from build123d import *

# Parameters (mm, degrees)
CUT_EXTRUDE_1_DEPTH = 5


with BuildPart() as part:
    # 草图1 → Revolve 587 (revolve)
    with BuildSketch(Plane.XY, mode=Mode.PRIVATE) as revolve_587_sk:
        Polygon((0, 0), (20, 0), (20, 2.75), (18.75, 4), (0.536, 4), (0, 3.464), align=None)
    revolve(revolve_587_sk.sketch.rotate(Axis((-0.277777778, 0, 0), (1, 0, 0)), 90), axis=Axis((-0.277777778, 0, 0), (1, 0, 0)))

    # 草图2 → 切除-拉伸1 (cut)
    with BuildSketch(Plane.ZY):
        Polygon((-1.154700538, -2), (1.154700538, -2), (2.309401077, 0), (1.154700538, 2), (-1.154700538, 2), (-2.309401077, 0), align=None)
    extrude(amount=-CUT_EXTRUDE_1_DEPTH, mode=Mode.SUBTRACT)

    # 草图4 → 切除-旋转2 (revolve, cut)
    with BuildSketch(Plane.XY, mode=Mode.PRIVATE) as cut_revolve_2_sk:
        Polygon((5, 2), (6.154700538, 0), (5, 0), align=None)
    revolve(cut_revolve_2_sk.sketch.rotate(Axis((-0.277777778, 0, 0), (1, 0, 0)), 90), axis=Axis((-0.277777778, 0, 0), (1, 0, 0)), mode=Mode.SUBTRACT)


solid = part.part
Geometry check sheet. Reference: the model listing, model coordinates, mm. A direction names the side the tool comes from. Round coordinates to 2 decimals unless told otherwise and drop trailing zeros. Loops run counter-clockwise (first coordinate to the right, second up) from the corner with the lowest first, then second, coordinate; pieces in that order, holes last.
Item 1: Thickness scan on line 1 (Y direction, x = 2.5, z = 1.5); line 2 (Y direction, x = 14, z = 1.5); line 3 (Z direction, x = 19.25, y = 0.5). Record the ranges inside material, lowest first.
Item 2: Cross-section at A-A on x = 4.25. Record the boundary of the cut face in (y, z), then the cut area to 3 significant figures.
Item 3: Access from +Z, -Z, +X, -X, +Y, -Y to the whole of each face (thin tool, end or side, straight path). Record for faces 4 (the flat face through (2, 2, 0)), 5 (the flat face through (20, 0, 0)).
Item 4: Gauge pin test, flat ends, axial feed: pin 1 (3 mm diameter, centred on x = 15, z = -2, fed in from -Y); pin 2 (1.5 mm diameter, centred on x = 8, z = -1.5, fed in from +Y); pin 3 (0.5 mm diameter, centred on y = 1.5, z = 1, fed in from -X). Record the tip position at first contact, or that the pin passes through.
Item 5: Mould release check, pull along Y, two halves, no side actions. Record for faces 1 (the flat face through (2.46, 0.99, 1.74)), 2 (the flat face through (0, 1, -2)), 3 (the cylindrical face through (9.516, 3.905, -0.867)): pulls with the +Y half, pulls with the -Y half, needs draft (parallel to the pull), parting line crosses it, or undercut.
Item 6: Cross-section at B-B on x = 14.25. Record the boundary of the cut face in (y, z), then the cut area to 3 significant figures.
Answer sheet:
1. line 1: y = -3.71 to -1.4, 1.4 to 3.71
1. line 2: y = -3.71 to 3.71
1. line 3: z = -3.46 to 3.46
2. outline: circle Ø8 at (0, 0); hole (-2, -1.15) - (0, -2.31) - (2, -1.15) - (2, 1.15) - (0, 2.31) - (-2, 1.15) - close
2. area: 36.4 mm2
3. face 4: -X
3. face 5: +Z, -Z, +X, +Y, -Y
4. pin 1: stops at y = -3.97
4. pin 2: stops at y = 3.93
4. pin 3: stops at x = 5
5. face 1: undercut
5. face 2: needs draft
5. face 3: parting line crosses it
6. outline: circle Ø8 at (0, 0)
6. area: 50.3 mm2
